Print and shaded views of the part. All mm, measured from the part's lowest x, y and z. A direction names the side the tool comes from. Round coordinates to 2 decimals unless told otherwise and drop trailing zeros. Order: outer loops, then holes, each group sorted by start corner. A loop starts at its lowest first (then second) coordinate and runs counter-clockwise, first axis right, second up. Notation, with made-up numbers: (82.25, 49.5) -> (108.25, 49.5) arc R16 cw to (108.25, 61.5) -> close; hole circle Ø10 at (-24, -34). An arc over 180 degrees is marked (long way). Answer as CSV lines item,"result".
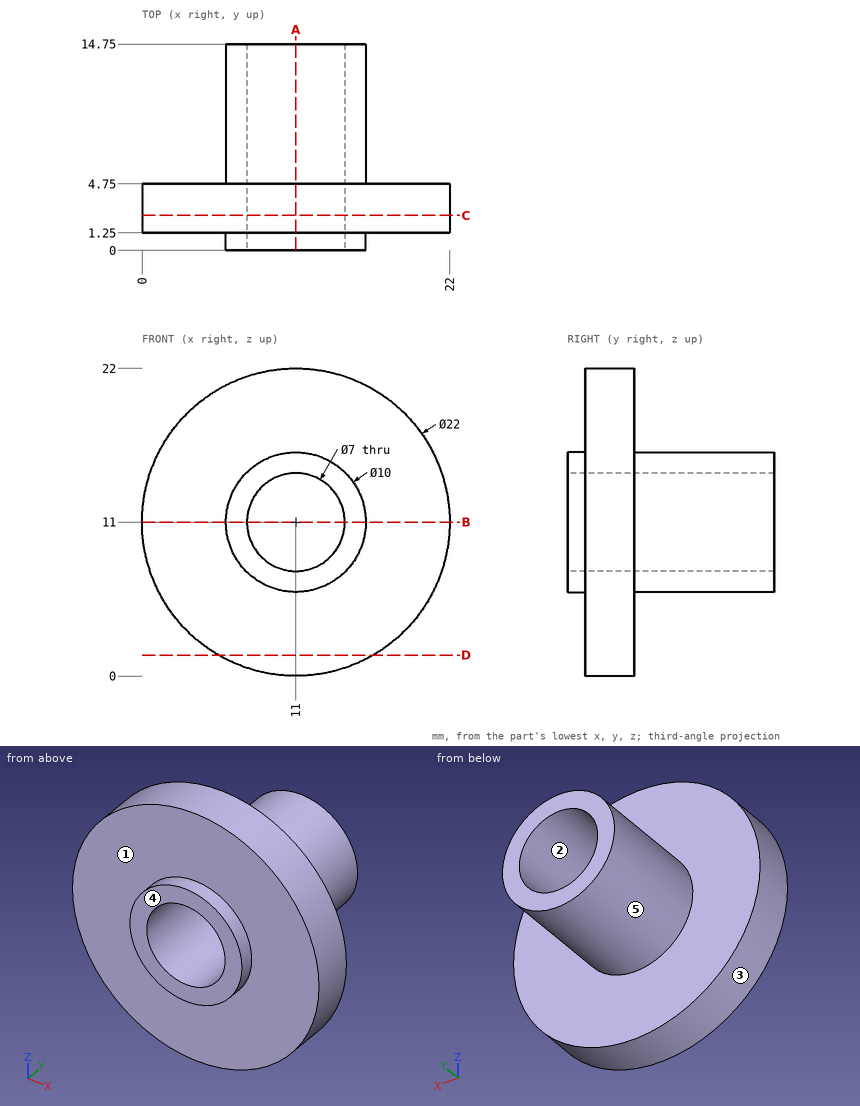
Q1. Flat gauge pins, fed straight in: pin 1 (2 mm diameter, centred on x = 9, z = 18, fed in from -Y); pin 2 (5 mm diameter, centred on x = 10.5, y = 8, fed in from +Z); pin 3 (4 mm diameter, centred on y = 3.5, z = 7.5, fed in from +X). Where does each tip first touch, or does it go through?
Checks:
pin 1,"y = 1.25"
pin 2,"z = 16"
pin 3,"x = 21.9"
Q2. Saw through at B-B (z = 11). Write the cut outline in (x, y), plus the area to 4 significant figures.
Checks:
outline,"(0, 1.25) -> (6, 1.25) -> (6, 0) -> (7.5, 0) -> (7.5, 14.75) -> (6, 14.75) -> (6, 4.75) -> (0, 4.75) -> close; (14.5, 0) -> (16, 0) -> (16, 1.25) -> (22, 1.25) -> (22, 4.75) -> (16, 4.75) -> (16, 14.75) -> (14.5, 14.75) -> close"
area,"86.25 mm²"
Q3. Wall check: L1, parallel to X at y = 6, z = 11; L2, parallel to X at y = 4.25, z = 11; L3, parallel to Y at x = 5, z = 17.25. Give the ranges that are in metal, low to high. Write a range as [from, to].
Checks:
L1,"[6, 7.5], [14.5, 16]"
L2,"[0, 7.5], [14.5, 22]"
L3,"[1.25, 4.75]"
Q4. Saw through at C-C (y = 2.5). Write the cut outline in (x, z), plus the area to 3 significant figures.
Checks:
outline,"circle Ø22 at (11, 11); hole circle Ø7 at (11, 11)"
area,"342 mm²"
Q5. Saw through at D-D (z = 1.5). Write the cut outline in (x, y).
Checks:
outline,"(5.45, 1.25) -> (16.55, 1.25) -> (16.55, 4.75) -> (5.45, 4.75) -> close"
Q6. Saw through at A-A (x = 11). Write the cut outline in (y, z), plus the area to 4 significant figures.
Checks:
outline,"(0, 6) -> (1.25, 6) -> (1.25, 0) -> (4.75, 0) -> (4.75, 6) -> (14.75, 6) -> (14.75, 7.5) -> (0, 7.5) -> close; (0, 14.5) -> (14.75, 14.5) -> (14.75, 16) -> (4.75, 16) -> (4.75, 22) -> (1.25, 22) -> (1.25, 16) -> (0, 16) -> close"
area,"86.25 mm²"
Q7. Mould opens along X. For the marked faces 1, 2 and 3 say: +X half, -X half, draft (parallel to the pull), parting line (faces both ways), or undercut.
Checks:
face 1,"draft"
face 2,"undercut"
face 3,"parting line"
Q8. Tool access for the marked faces 4 and 5: list every direction of +Z, -Z, +X, -X, +Y, -Y with a clear straight run to the whole face (end or side of a thin tool).
Checks:
face 4,"+Z, -Z, +X, -X, -Y"
face 5,"+Y"
